The listing builds one solid part. Answer for the finished solid, in the listing's coordinates (mm). A direction names the side the tool comes from. Round coordinates to 2 decimals unless told otherwise and drop trailing zeros. Loops run counter-clockwise (first coordinate to the right, second up) from the corner with the lowest first, then second, coordinate; pieces in that order, holes last. Notation, with made-up numbers: (5.25, 39) -> (23.25, 39) arc R27 ccw to (23.25, 63) -> close; hole circle Ø5 at (-14, -35). An arc over 180 degrees is marked (long way). Use a Markdown table: item, result. Add a question column.
Q1. Consider line 1 (X direction, y = -134, z = 134); line 2 (Y direction, x = 66, z = 11); line 3 (Z direction, x = 98, y = 110). Determine where each line is inside the solid, lowest interval first.
Q2. Which of the six approach directions +Z, -Z, +X, -X, +Y, -Y give full straight-line access (tool end or side, diameter ignored) to faces 5 (the flat face through (260, 3, 145)), 6 (the flat face through (-250, -3, 102)), 7 (the flat face through (-89, 30, 2))?
Q3. Section D-D on x = -218 is taken. Give the vertices of the cut face in (y, z), then the cut area to 3 significant figures.
Q4. Section C-C on z = 92 is taken. Give the vertices of the cut face in (x, y), then the cut area to 3 significant figures.
Q5. For a pull along Y with two mould halves and no side action, classify faces 1 (the flat face through (-248, -3, 105)), 2 (the flat face through (250, -3, 102)), 3 (the flat face through (-3, 198, 75)), 4 (the flat face through (-4, -200, 93)) as released by +Y, released by -Y, zero draft, split by the parting line, or undercut.
Q6. Section B-B on y = 130 is taken. Give the vertices of the cut face in (x, z).
Q7. Given pin 1 Ø22 at (x, y) = (257, 41.5) entering from -Z; pin 2 Ø5 at (y, z) = (130.5, 87) entering from -X; pin 3 Ø1.5 at (x, y) = (-120, 130.5) entering from +Z, each flat-ended and moving along its own axis, determine where each tip first touches the part or whether it passes through.
Q8. Section A-A on x = -54 is taken. Give the vertices of the cut face in (y, z).
from build123d import *

# Parameters (mm, degrees)
SKETCH_1_W          = 500
SKETCH_1_H          = 400
EXTRUDE_1_DEPTH     = 150
CUT_EXTRUDE_1_DEPTH = 495.974746831
SHELL_1_T           = -2
SKETCH_2_W          = 20
SKETCH_2_H          = 400
EXTRUDE_2_DEPTH     = 5
SKETCH_4_W          = 175
SKETCH_4_H          = 380
CUT_EXTRUDE_2_DEPTH = 368.15664232


with BuildPart() as part:
    # 草图1 → 凸台-拉伸1 (new body)
    with BuildSketch(Plane.XY):
        Rectangle(SKETCH_1_W, SKETCH_1_H)
    extrude(amount=EXTRUDE_1_DEPTH)

    # 草图3 → 切除-拉伸1 (cut, through all)
    with BuildSketch(Plane.XZ.offset(200)):
        Polygon((-100, 0), (-250, 60), (-250, 0), align=None)
        Polygon((250, 60), (100, 0), (250, 0), align=None)
    extrude(amount=-CUT_EXTRUDE_1_DEPTH, mode=Mode.SUBTRACT)

    # 抽壳1
    shell_1_openings = [part.faces().sort_by_distance(p)[0] for p in [
        (0, 0, 150),
    ]]
    offset(amount=SHELL_1_T, openings=shell_1_openings, kind=Kind.INTERSECTION)

    # 草图2 → 凸台-拉伸2 (add)
    with BuildSketch(Plane.XY.offset(150)):
        with Locations((-260, 0)):
            Rectangle(SKETCH_2_W, SKETCH_2_H)
        with Locations((260, 0)):
            Rectangle(SKETCH_2_W, SKETCH_2_H)
    extrude(amount=-EXTRUDE_2_DEPTH)

    # 草图4 → 切除-拉伸2 (cut, through all)
    with BuildSketch(Plane.XY.offset(2)):
        Rectangle(SKETCH_4_W, SKETCH_4_H)
    extrude(amount=-CUT_EXTRUDE_2_DEPTH, mode=Mode.SUBTRACT)


solid = part.part
Checked values:
| question | item | result |
|---|---|---|
| 1 | line 1 | x = -250 to -248, 248 to 250 |
| 1 | line 2 | y = -200 to -198, 198 to 200 |
| 1 | line 3 | z = 0 to 2 |
| 2 | face 5 | -Z, +X, +Y, -Y |
| 2 | face 6 | -Z, -X, +Y, -Y |
| 2 | face 7 | +Z |
| 3 | outline | (-200, 47.2) -> (200, 47.2) -> (200, 150) -> (198, 150) -> (198, 49.35) -> (-198, 49.35) -> (-198, 150) -> (-200, 150) -> close |
| 3 | area | 1,260 mm2 |
| 4 | outline | (-250, -200) -> (250, -200) -> (250, 200) -> (-250, 200) -> close; hole (-248, -198) -> (248, -198) -> (248, 198) -> (-248, 198) -> close |
| 4 | area | 3,580 mm2 |
| 5 | face 1 | undercut |
| 5 | face 2 | zero draft |
| 5 | face 3 | undercut |
| 5 | face 4 | released by -Y |
| 6 | outline | (-270, 145) -> (-250, 145) -> (-250, 60) -> (-100, 0) -> (-87.5, 0) -> (-87.5, 2) -> (-99.61, 2) -> (-248, 61.35) -> (-248, 150) -> (-270, 150) -> close; (87.5, 0) -> (100, 0) -> (250, 60) -> (250, 145) -> (270, 145) -> (270, 150) -> (248, 150) -> (248, 61.35) -> (99.61, 2) -> (87.5, 2) -> close |
| 7 | pin 1 | stops at z = 58.4 |
| 7 | pin 2 | stops at x = -250 |
| 7 | pin 3 | stops at z = 10.45 |
| 8 | outline | (-200, 0) -> (-190, 0) -> (-190, 2) -> (-198, 2) -> (-198, 150) -> (-200, 150) -> close; (190, 0) -> (200, 0) -> (200, 150) -> (198, 150) -> (198, 2) -> (190, 2) -> close |
